from build123d import *

# Parameters (mm, degrees)
FLANGE_PROFILE_SKETCH_R  = 5
FLANGE_PLATE_15MM_DEPTH  = 15
SADDLE_BODY_100MM_DEPTH  = 100
SUPPORT_BLOCK_SKETCH_R   = 10
SUPPORT_BLOCK_63MM_DEPTH = 63
SLOT_CUT_DEPTH           = 167.282891483
SLOT_CUT_DEPTH_BACK      = 167.282891483
SLOT_CUT_SKETCH_W        = 45.5
SLOT_CUT_SKETCH_H        = 45
CROSS_HOLE_SKETCH_R      = 5
CROSS_HOLE_DEPTH         = 63


with BuildPart() as part:
    # Flange Profile Sketch → Flange Plate 15mm (new body)
    with BuildSketch(Plane.XY):
        with BuildLine():
            ThreePointArc((-12, 100), (0, 88), (12, 100))
            Line((12, 100), (15, 100))
            Line((15, 100), (15, 125))
            Line((15, 125), (30, 125))
            ThreePointArc((30, 125), (37.071067812, 122.071067812), (40, 115))
            Line((40, 115), (40, 25))
            ThreePointArc((40, 25), (0, 65), (-40, 25))
            Line((-40, 25), (-40, 115))
            ThreePointArc((-40, 115), (-37.071067812, 122.071067812), (-30, 125))
            Line((-30, 125), (-15, 125))
            Line((-15, 125), (-15, 100))
            Line((-15, 100), (-12, 100))
        make_face()
        with Locations((-30, 115)):
            Circle(FLANGE_PROFILE_SKETCH_R, mode=Mode.SUBTRACT)
        with Locations((30, 115)):
            Circle(FLANGE_PROFILE_SKETCH_R, mode=Mode.SUBTRACT)
    extrude(amount=FLANGE_PLATE_15MM_DEPTH)

    # Sketch1_4 → Saddle Body 100mm (add)
    with BuildSketch(Plane.XY):
        with BuildLine():
            ThreePointArc((30, 25), (0, 55), (-30, 25))
            Line((-30, 25), (-30, 10))
            Line((-30, 10), (-20, 10))
            Line((-20, 10), (-20, 0))
            Line((-20, 0), (-45, 0))
            Line((-45, 0), (-45, 25))
            Line((-45, 25), (-40, 25))
            ThreePointArc((-40, 25), (0, 65), (40, 25))
            Line((40, 25), (45, 25))
            Line((45, 25), (45, 0))
            Line((45, 0), (20, 0))
            Line((20, 0), (20, 10))
            Line((20, 10), (30, 10))
            Line((30, 10), (30, 25))
        make_face()
    extrude(amount=SADDLE_BODY_100MM_DEPTH)

    # Support Block Sketch → Support Block 63mm (add)
    with BuildSketch(Plane.XY.offset(15)):
        with BuildLine():
            Line((-19.275776393, 105.333333333), (-38.551552786, 35.666666667))
            ThreePointArc((-38.551552786, 35.666666667), (0, 65), (38.551552786, 35.666666667))
            Line((38.551552786, 35.666666667), (19.275776393, 105.333333333))
            ThreePointArc((19.275776393, 105.333333333), (0, 120), (-19.275776393, 105.333333333))
        make_face()
        with Locations((0, 100)):
            Circle(SUPPORT_BLOCK_SKETCH_R, mode=Mode.SUBTRACT)
    extrude(amount=SUPPORT_BLOCK_63MM_DEPTH)

    # Slot Cut Sketch → Slot Cut (cut, two sides: drawn at the far end of the back side and taken through both)
    with BuildSketch(Plane(origin=(0, 0, 0), x_dir=(0, 0, -1), z_dir=(1, 0, 0)).offset(-SLOT_CUT_DEPTH_BACK)):
        with Locations((-37.75, 102.5)):
            Rectangle(SLOT_CUT_SKETCH_W, SLOT_CUT_SKETCH_H)
    extrude(amount=SLOT_CUT_DEPTH + SLOT_CUT_DEPTH_BACK, mode=Mode.SUBTRACT)

    # Cross Hole Sketch → Cross Hole (cut)
    with BuildSketch(Plane(origin=(0, 80, 0), x_dir=(1, 0, 0), z_dir=(0, 1, 0))):
        with Locations(Location((0, -40, 0), (0, 0, 270))):
            Circle(CROSS_HOLE_SKETCH_R)
    extrude(amount=-CROSS_HOLE_DEPTH, mode=Mode.SUBTRACT)


solid = part.part
Verification items for the finished model (mm, model axes). A direction names the side the tool comes from. Give positions to 0.01 mm unless a question says otherwise; leave off trailing zeros. Write each loop counter-clockwise with the first axis right and the second up, starting at its lowest first coordinate (ties: lowest second). Pieces come first, ordered by that corner, then holes.
(1) Cross-section at D-D (z = 21). Enter the section's corners in (x, y).
(2) Access from +Z, -Z, +X, -X, +Y, -Y to the whole of each face (thin tool, end or side, straight path). Record for faces 5 (the face through (0, 120, 69)), 6 (the face through (-25, 10, 49)), 7 (the face through (-15, 113, 7)).
(3) Cross-section at C-C (y = 95). Enter the section's corners in (x, z).
(4) Cross-section at A-A (z = 74). Enter the section's corners in (x, y), plus the area to 3 significant figures.
(5) Mould release check, pull along Y, two halves, no side actions. Record for faces 1 (the face through (40, 71, 7)), 2 (the face through (-34, 118, 7)), 3 (the face through (33, 0, 49)), 4 (the face through (-14, 100, 7)): +Y half, -Y half, draft (parallel to the pull), parting line (faces both ways), or undercut.
(6) Material ranges on line 1 (Y direction, x = 0, z = 74); line 2 (Z direction, x = 0, y = 72); line 3 (Z direction, x = 0, y = 61), recorded low to high.
(7) Cross-section at B-B (z = 40). Enter the section's corners in (x, y), plus the area to 3 significant figures.
(8) Gauge pin test, flat ends, axial feed: pin 1 (3 mm diameter, centred on x = -19, z = 54, fed in from +Y); pin 2 (12 mm diameter, centred on x = 20, y = 105.5, fed in from +Z); pin 3 (13 mm diameter, centred on x = 30, y = 115, fed in from +Z). Record the tip position at first contact, or that the pin passes through.
Worked out:
1. outline: (-45, 0) - (-20, 0) - (-20, 10) - (-30, 10) - (-30, 25) arc R30 cw to (30, 25) - (30, 10) - (20, 10) - (20, 0) - (45, 0) - (45, 25) - (40, 25) arc R40 ccw to (38.55, 35.67) - (26.29, 80) - (-26.29, 80) - (-38.55, 35.67) arc R40 ccw to (-40, 25) - (-45, 25) - close
2. face 5: +Z, +Y
2. face 6: +Z, -Z
2. face 7: -Z, +Y
3. outline: (-40, 0) - (-10.91, 0) - (-10.91, 15) - (-40, 15) - close; (-22.13, 60.5) - (-8.66, 60.5) - (-8.66, 78) - (-22.13, 78) - close; (8.66, 60.5) - (22.13, 60.5) - (22.13, 78) - (8.66, 78) - close; (10.91, 0) - (40, 0) - (40, 15) - (10.91, 15) - close
4. outline: (-45, 0) - (-20, 0) - (-20, 10) - (-30, 10) - (-30, 25) arc R30 cw to (30, 25) - (30, 10) - (20, 10) - (20, 0) - (45, 0) - (45, 25) - (40, 25) arc R40 ccw to (38.55, 35.67) - (19.28, 105.33) arc R20 ccw to (-19.28, 105.33) - (-38.55, 35.67) arc R40 ccw to (-40, 25) - (-45, 25) - close; hole circle Ø20 at (0, 100)
4. area: 4,510 mm2
5. face 1: draft
5. face 2: undercut
5. face 3: -Y half
5. face 4: +Y half
6. line 1: y = 55 to 90, 110 to 120
6. line 2: z = 0 to 35, 45 to 78
6. line 3: z = 0 to 35, 45 to 100
7. outline: (-45, 0) - (-20, 0) - (-20, 10) - (-30, 10) - (-30, 25) arc R30 cw to (-5, 54.58) - (-5, 80) - (-26.29, 80) - (-38.55, 35.67) arc R40 ccw to (-40, 25) - (-45, 25) - close; (5, 54.58) arc R30 cw to (30, 25) - (30, 10) - (20, 10) - (20, 0) - (45, 0) - (45, 25) - (40, 25) arc R40 ccw to (38.55, 35.67) - (26.29, 80) - (5, 80) - close
7. area: 3,000 mm2
8. pin 1: stops at y = 80
8. pin 2: stops at z = 78
8. pin 3: stops at z = 15
